Could you check a few things on this model? Use its own coordinates, in mm. A direction names the side the tool comes from. Coordinates: 2 decimals unless noted, no trailing zeros. Loops run counter-clockwise (first coordinate to the right, second up) from the corner with the lowest first, then second, coordinate; pieces in that order, holes last.
1) For faces 1 (the face through (8, 0, -20.5)), 2 (the face through (73.3, 7.7, -10.1)), which set-ups out of +Z, -Z, +X, -X, +Y, -Y let a thin tool reach every point of the face, with its end or its side?
2) If I drill on line 1 along X through (y, z) = (-14, -6.5); line 2 along Y through (x, z) = (103.5, 5.5); line 3 along Z through (x, y) = (36.5, 11), over which ranges is the centre line in solid material (lowest first)?
3) Imagine slicing it at A-A on x = 59.5. Please give me the cut outline in (y, z), plus the area to 3 significant figures.
4) Will these pins go through, and if not, where does the flat tip stop? P1, Ø10, axis at x = 30.5, y = -8.5, coming from the -Z side; P2, Ø3, axis at y = -7.5, z = 13.5, coming from the +X side; P3, Ø5, axis at x = 82.5, y = -2, coming from the +Z side.
```python
from build123d import *

# Parameters (mm, degrees)
BASE_EXTRUDE_DEPTH = 17
CHAMFER_2_SIZE     = 2.5
FILLET_2_R         = 2.4


with BuildPart() as part:
    # Sketch1 → Base-Extrude (new body)
    with BuildSketch(Plane(origin=(0, 0, 0), x_dir=(0, 0, -1), z_dir=(1, 0, 0))):
        Polygon((20.5, 11.835680518), (20.5, -11.835680518), (0, -23.671361037), (-20.5, -11.835680518), (-20.5, 11.835680518), (0, 23.671361037), align=None)
    extrude(amount=BASE_EXTRUDE_DEPTH)

    # Sketch2 → Boss-Revolve1 (revolve)
    with BuildSketch(Plane.XY, mode=Mode.PRIVATE) as boss_revolve1_sk:
        Polygon((0, 0), (131.3, 0), (131.3, 10.902), (131.3, 12.7), (27.8072, 12.7), (0, 12.7), align=None)
    revolve(boss_revolve1_sk.sketch.rotate(Axis((0, 0, 0), (1, 0, 0)), 90), axis=Axis((0, 0, 0), (1, 0, 0)))

    # Sketch3 → Cut-Revolve1 (revolve, cut)
    with BuildSketch(Plane.XY):
        Polygon((0, 20.5), (4.717737494, 28.671361037), (4.717737494, 33.671361037), (-10, 33.671361037), (-10, 20.5), align=None)
    revolve(axis=Axis((0, 0, 0), (1, 0, 0)), mode=Mode.SUBTRACT)

    # Chamfer 2
    chamfer_2_edges = [part.edges().sort_by_distance(p)[0] for p in [
        (131.3, 0, -12.7),
    ]]
    chamfer(chamfer_2_edges, length=CHAMFER_2_SIZE)

    # Fillet 2
    fillet_2_edges = [part.edges().sort_by_distance(p)[0] for p in [
        (17, 0, -12.7),
    ]]
    fillet(fillet_2_edges, radius=FILLET_2_R)


solid = part.part
```
Filled in:
1. face 1: -Z, +X, -X, +Y, -Y
1. face 2: +X
2. line 1: x = 0 to 17
2. line 2: y = -11.45 to 11.45
2. line 3: z = -6.35 to 6.35
3. outline: circle Ø25.4 at (0, 0)
3. area: 507 mm2
4. P1: stops at z = -12.21
4. P2: stops at x = 17.3
4. P3: stops at z = 12.7
